from build123d import *

# Parameters (mm, degrees)
SKETCH_1_W            = 70
SKETCH_1_H            = 80
EXTRUDE_1_DEPTH       = 12
CHAMFER_1_SIZE        = 1
HOLE_WIZARD_7_0_7_1_D = 7
HOLE_WIZARD_M6_1_D    = 5


with BuildPart() as part:
    # 草图1 → 凸台-拉伸1 (new body)
    with BuildSketch(Plane.XY):
        with Locations((35, -40)):
            Rectangle(SKETCH_1_W, SKETCH_1_H)
    extrude(amount=EXTRUDE_1_DEPTH)

    # 倒角1
    chamfer_1_edges = [part.edges().sort_by_distance(p)[0] for p in [
        (0, 0, 6),
        (70, 0, 6),
        (70, -80, 6),
        (0, -80, 6),
    ]]
    chamfer(chamfer_1_edges, length=CHAMFER_1_SIZE)

    # Ø7.0 (7) 直径孔1 (through all)
    with Locations(Plane(origin=(0, 0, 0), x_dir=(-1, 0, 0), z_dir=(0, 0, -1))):
        with Locations((-7, -73), (-7, -7), (-63, -73), (-63, -7)):
            Hole(HOLE_WIZARD_7_0_7_1_D / 2)

    # M6 螺纹孔1 (through all)
    with Locations(Plane(origin=(0, 0, 0), x_dir=(-1, 0, 0), z_dir=(0, 0, -1))):
        with Locations((-57, -32.5), (-57, -47.5), (-13, -47.5), (-13, -32.5)):
            Hole(HOLE_WIZARD_M6_1_D / 2)


solid = part.part
Here's how the part is built. I have some questions about the finished solid (model axes, mm). Give positions to 0.01 mm unless a question says otherwise; leave off trailing zeros. Order: outer loops, then holes, each group sorted by start corner. A loop starts at its lowest first (then second) coordinate and runs counter-clockwise, first axis right, second up. Notation, with made-up numbers: M 10.5,-2 L 18.5,-2 A26 cw 18.5,15 Z; hole C 29.25,50.5 d11. An arc over 180 degrees is marked long. Answer as a JSON object with one key per item and string values. Group by question number.
1) Suppose I cut it at C-C, the plane x = 13. Write out the boundary of the cut face in (y, z), plus the area to 3 significant figures.
2) Please list where these lines run through material, in increasing order: L1, parallel to Y at x = 57, z = 3.5; L2, parallel to Y at x = 63, z = 4; L3, parallel to X at y = -5, z = 9.75. Write a range as [from, to].
3) We'd pull the mould along X, two halves only. Please class faces 1 (the flat face through (70, -41, 6)), 2 (the cylindrical face through (60.2, -75.1, 6.1)), 3 (the flat face through (35, -80, 6)): pulls with the +X half, pulls with the -X half, needs draft (parallel to the pull), parting line crosses it, or undercut.
4) Suppose I cut it at A-A, the plane y = -32.5. Write out the boundary of the cut face in (x, z).
5) Suppose I cut it at B-B, the plane z = 10. Count the separate pieces of the cut face and the enclosed holes in it, plus the area to 3 significant figures.
Results found:
{
 "1": {"outline": "M -80,0 L -50,0 L -50,12 L -80,12 Z; M -45,0 L -35,0 L -35,12 L -45,12 Z; M -30,0 L 0,0 L 0,12 L -30,12 Z", "area": "840 mm²"},
 "2": {"L1": "[-80, -50], [-45, -35], [-30, 0]", "L2": "[-80, -76.5], [-69.5, -10.5], [-3.5, 0]", "L3": "[0, 4.13], [9.87, 60.13], [65.87, 70]"},
 "3": {"face 1": "pulls with the +X half", "face 2": "undercut", "face 3": "needs draft"},
 "4": {"outline": "M 0,0 L 10.5,0 L 10.5,12 L 0,12 Z; M 15.5,0 L 54.5,0 L 54.5,12 L 15.5,12 Z; M 59.5,0 L 70,0 L 70,12 L 59.5,12 Z"},
 "5": {"separate pieces": "1", "enclosed holes": "8", "area": "5,370 mm²"}
}
